from build123d import *
from build123d.topology import SkipClean

# Parameters (mm, degrees)
U_BASE_DEPTH             = 20
UPRIGHT_WEB_DEPTH        = 50
CYLINDER_50_SKETCH_R     = 25
CYLINDER_50_DEPTH        = 50
WEB_CLEARANCE_CUT_DEPTH  = 50
SIDE_RELIEF_CUT_SKETCH_W = 18
SIDE_RELIEF_CUT_SKETCH_H = 35
SIDE_RELIEF_CUT_DEPTH    = 50
BASE_SLOT_CUT_SKETCH_W   = 50
BASE_SLOT_CUT_SKETCH_H   = 50
BASE_SLOT_CUT_DEPTH      = 10
WEB_SLOT_CUT_SKETCH_W    = 5
WEB_SLOT_CUT_SKETCH_H    = 50
WEB_SLOT_CUT_DEPTH       = 10
END_START                = 20
END_BOSS_A_SKETCH_R      = 25
END_BOSS_A_50_DEPTH      = 20
END_BOSS_B_SKETCH_R      = 25
END_BOSS_B_50_DEPTH      = 20
END_SLOT_A_DEPTH         = 10
END_START_2              = -10
END_SLOT_B_DEPTH         = 10


with BuildPart() as part:
    # U Base Profile Sketch → U Base (new body)
    with BuildSketch(Plane(origin=(0, 0, 0), x_dir=(0, 0, -1), z_dir=(1, 0, 0))):
        Polygon((25, 0), (-25, 0), (-25, 20), (-9, 20), (-9, 6), (9, 6), (9, 20), (25, 20), align=None)
    extrude(amount=U_BASE_DEPTH)

    # Upright Web Sketch → Upright Web (add)
    with BuildSketch(Plane.ZY):
        Polygon((-9, 20), (-9, 65), (9, 65), (9, 20), (25, 20), (25, 70), (-25, 70), (-25, 20), align=None)
        Polygon((25, 20), (9, 20), (9, 6), (-9, 6), (-9, 20), (-25, 20), (-25, 0), (25, 0), align=None)
    extrude(amount=UPRIGHT_WEB_DEPTH)

    # Cylinder Ø50 Sketch → Cylinder Ø50 (add)
    with BuildSketch(Plane.XY.offset(25)):
        with Locations((-25, 55)):
            Circle(CYLINDER_50_SKETCH_R)
    extrude(amount=-CYLINDER_50_DEPTH)

    # Web Clearance Cut Sketch → Web Clearance Cut (cut)
    with SkipClean():  # the faces are left unmerged after this step: merging them gives an invalid solid
        with BuildSketch(Plane.XY.offset(25)):
            with BuildLine():
                Line((-50, 70), (-50, 55))
                ThreePointArc((-50, 55), (-48.717082, 62.905694), (-45, 70))
                Line((-45, 70), (-50, 70))
            make_face()
            with BuildLine():
                ThreePointArc((-5, 70), (-1.282918, 62.905694), (0, 55))
                Line((0, 55), (0, 70))
                Line((0, 70), (-5, 70))
            make_face()
        extrude(amount=-WEB_CLEARANCE_CUT_DEPTH, mode=Mode.SUBTRACT)

    # Side Relief Cut Sketch → Side Relief Cut (cut)
    with SkipClean():  # the faces are left unmerged after this step: merging them gives an invalid solid
        with BuildSketch(Plane(origin=(0, 0, 0), x_dir=(0, 0, -1), z_dir=(1, 0, 0))):
            with Locations((0, 37.5)):
                Rectangle(SIDE_RELIEF_CUT_SKETCH_W, SIDE_RELIEF_CUT_SKETCH_H)
        extrude(amount=-SIDE_RELIEF_CUT_DEPTH, mode=Mode.SUBTRACT)

    # Base Slot Cut Sketch → Base Slot Cut (cut)
    with SkipClean():  # the faces are left unmerged after this step: merging them gives an invalid solid
        with BuildSketch(Plane(origin=(0, 0, 0), x_dir=(0, 0, -1), z_dir=(1, 0, 0))):
            with Locations((0, 45)):
                Rectangle(BASE_SLOT_CUT_SKETCH_W, BASE_SLOT_CUT_SKETCH_H)
        extrude(amount=-BASE_SLOT_CUT_DEPTH, mode=Mode.SUBTRACT)

    # Web Slot Cut Sketch → Web Slot Cut (cut)
    with SkipClean():  # the faces are left unmerged after this step: merging them gives an invalid solid
        with BuildSketch(Plane.XZ.offset(-70)):
            with Locations((-7.5, 0)):
                Rectangle(WEB_SLOT_CUT_SKETCH_W, WEB_SLOT_CUT_SKETCH_H)
        extrude(amount=-WEB_SLOT_CUT_DEPTH, mode=Mode.SUBTRACT)

    # End Boss A Sketch → End Boss A Ø50 (add)
    with BuildSketch(Plane.XY.offset(25).offset(END_START)):
        with Locations((-25, 55)):
            Circle(END_BOSS_A_SKETCH_R)
    extrude(amount=-END_BOSS_A_50_DEPTH)

    # End Boss B Sketch → End Boss B Ø50 (add)
    with BuildSketch(Plane(origin=(0, 0, -25), x_dir=(-1, 0, 0), z_dir=(0, 0, -1))):
        with Locations(Location((25, 55, 0), (0, 0, 180))):
            Circle(END_BOSS_B_SKETCH_R)
    extrude(amount=END_BOSS_B_50_DEPTH)

    # End Slot A Sketch → End Slot A (cut)
    with BuildSketch(Plane.XY.offset(45)):
        with BuildLine():
            Line((-46.354157, 68), (-3.645843, 68))
            ThreePointArc((-3.645843, 68), (-25, 80), (-46.354157, 68))
        make_face()
    extrude(amount=-END_SLOT_A_DEPTH, mode=Mode.SUBTRACT)

    # End Slot B Sketch → End Slot B (cut)
    with BuildSketch(Plane(origin=(0, 0, -45), x_dir=(-1, 0, 0), z_dir=(0, 0, -1)).offset(END_START_2)):
        with BuildLine():
            Line((3.645843, 68), (46.354157, 68))
            ThreePointArc((46.354157, 68), (25, 80), (3.645843, 68))
        make_face()
    extrude(amount=END_SLOT_B_DEPTH, mode=Mode.SUBTRACT)


solid = part.part
Could you check a few things on this model? Use its own coordinates, in mm. A direction names the side the tool comes from. Give positions to 0.01 mm unless a question says otherwise; leave off trailing zeros. Loops run counter-clockwise (first coordinate to the right, second up) from the corner with the lowest first, then second, coordinate; pieces in that order, holes last. Notation, with made-up numbers: M 11.5,-10 L 56.5,-10 A17 ccw 56.5,15 Z; hole C 9,-18 d7. An arc over 180 degrees is marked long. Answer as a JSON object with one key per item and string values.
Q1. Suppose I cut it at C-C, the plane z = -23.5. List the corners of the cut face in (x, y) for me, plus the area to 3 significant figures.
Values found:
{"outline": "M -50,0 L 20,0 L 20,20 L -10,20 L -10,75 A25 ccw -45,70 A25 ccw -50,55 Z", "area": "3,640 mm²"}
Q2. If I drill on probe 1 along Z at (x, y) = (-25.5, 34); probe 2 along Y at (x, z) = (-24, 4); probe 3 along Z at (x, y) = (-39.5, 17), over which ranges is the centre line in solid material (lowest first)? Write a range as [from, to].
Values found:
{"probe 1": "z = [-45, -9], [9, 45]", "probe 2": "y = [0, 6], [55, 79.98]", "probe 3": "z = [-25, -9], [9, 25]"}
Q3. Suppose I cut it at B-B, the plane y = 50. List the corners of the cut face in (x, z) for me.
Values found:
{"outline": "M -50,-25 L -49.49,-25 L -49.49,-45 L -0.51,-45 L -0.51,-25 L -10,-25 L -10,-9 L -50,-9 Z; M -50,9 L -10,9 L -10,25 L -0.51,25 L -0.51,45 L -49.49,45 L -49.49,25 L -50,25 Z"}
Q4. For faces 1 (the flat face through (-6, 55, -25)), 2 (the flat face through (-25, 73, 35)), 3 (the flat face through (-25, 68, -40)), 4 (the flat face through (-15, 6, 0)), 5 (the flat face through (-25, 49, 45)), which set-ups out of +Z, -Z, +X, -X, +Y, -Y let a thin tool reach every point of the face, with its end or its side?
Values found:
{"face 1": "+X, +Y", "face 2": "+Z, +X, -X, +Y", "face 3": "-Z, +X, -X, +Y", "face 4": "+X, -X", "face 5": "+Z, +X, -X, +Y, -Y"}
Q5. Suppose I cut it at A-A, the plane x = -25. List the corners of the cut face in (y, z) for me, plus the area to 3 significant figures.
Values found:
{"outline": "M 0,-25 L 30,-25 L 30,-45 L 68,-45 L 68,-35 L 80,-35 L 80,35 L 68,35 L 68,45 L 30,45 L 30,25 L 0,25 Z; hole M 6,-9 L 55,-9 L 55,9 L 6,9 Z", "area": "4,880 mm²"}
Q6. If we mould it in two halves opening along Z, with no side actions, what happens to faces 6 (the flat face through (5, 20, 17)), 7 (the flat face through (-10, 60, 0)), 8 (the flat face through (-25, 53, -45))? For each: pulls with the +Z half, pulls with the -Z half, needs draft (parallel to the pull), parting line crosses it, or undercut.
Values found:
{"face 6": "needs draft", "face 7": "undercut", "face 8": "pulls with the -Z half"}
Q7. Suppose I cut it at D-D, the plane z = 3. List the corners of the cut face in (x, y) for me.
Values found:
{"outline": "M -50,0 L 20,0 L 20,6 L -50,6 Z; M -50,55 L -10,55 L -10,75 A25 ccw -45,70 A25 ccw Z"}
Q8. For P1, Ø5, axis at x = 8, z = 17, coming from the +Y side; P2, Ø12, axis at x = -4, y = 13, coming from the +Z side; P3, Ø6, axis at x = -18, y = 75, coming from the +Z side; P4, Ø20, axis at x = -33, z = -4.5, coming from the -Y side, each with a flat end and sliding along its axis, tell me the tip position at first contact or that it passes through.
Values found:
{"P1": "stops at y = 20", "P2": "stops at z = 25", "P3": "stops at z = 35", "P4": "stops at y = 0"}
